Part model, mm, in its own coordinate system. Round coordinates to 2 decimals unless told otherwise and drop trailing zeros. Loops run counter-clockwise (first coordinate to the right, second up) from the corner with the lowest first, then second, coordinate; pieces in that order, holes last.
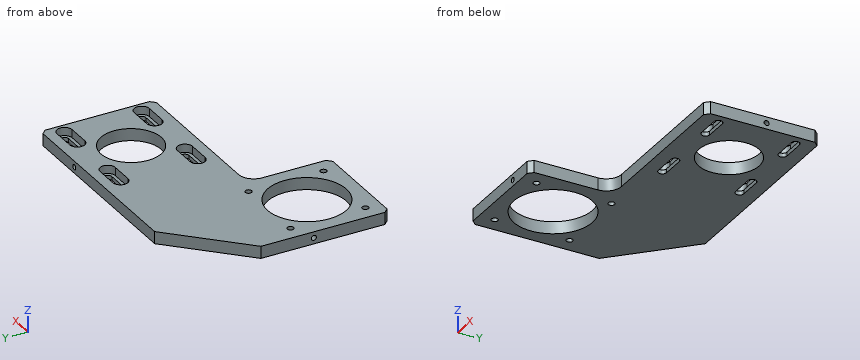
from build123d import *

# Parameters (mm, degrees)
SKETCH_2_W                     = 180
SKETCH_2_H                     = 130
EXTRUDE_1_DEPTH                = 4
SKETCH_3_W                     = 110
SKETCH_3_H                     = 55
CUT_EXTRUDE_1_DEPTH            = 8
SKETCH_4_R                     = 26
CUT_EXTRUDE_2_DEPTH            = 8
HOLE_WIZARD_M5_1_D             = 4.2
HOLE_WIZARD_M5_1_DEPTH         = 12.4
HOLE_WIZARD_M5_1_TIP           = 1.2618073
SKETCH_7_R                     = 20
CUT_EXTRUDE_3_DEPTH            = 8
HOLE_WIZARD_M4_1_D             = 3.3
HOLE_WIZARD_M4_1_DEPTH         = 12
HOLE_WIZARD_M4_1_TIP           = 0.991420021
HOLE_WIZARD_M4_2_D             = 3.3
HOLE_WIZARD_M4_2_DEPTH         = 12
HOLE_WIZARD_M4_2_TIP           = 0.991420021
CHAMFER_1_SIZE                 = 45
CHAMFER_2_SIZE                 = 3
FILLET_1_R                     = 10
HOLE_WIZARD_M5_1_2_D           = 5.5
HOLE_WIZARD_M5_1_2_DEPTH       = 10.1
HOLE_WIZARD_M5_1_2_CBORE_D     = 10
HOLE_WIZARD_M5_1_2_CBORE_DEPTH = 5.4
HOLE_WIZARD_M5_1_2_TIP         = 1.652366702
CUT_EXTRUDE_6_DEPTH            = 112.30588484
CUT_EXTRUDE_7_DEPTH            = 5.4
PATTERN_LINEAR_1_COUNT         = 2
PATTERN_LINEAR_1_PITCH         = 51
PATTERN_LINEAR_1_COUNT_DIR2    = 2
PATTERN_LINEAR_1_PITCH_DIR2    = 51
HOLE_WIZARD_M4_3_D             = 3.3
HOLE_WIZARD_M4_3_DEPTH         = 10.1
HOLE_WIZARD_M4_3_TIP           = 0.991420021
HOLE_WIZARD_M4_4_D             = 3.3
HOLE_WIZARD_M4_4_DEPTH         = 10.1
HOLE_WIZARD_M4_4_TIP           = 0.991420021


with BuildPart() as part:
    # 草图2 → 凸台-拉伸1 (new, symmetric)
    with BuildSketch(Plane.XY):
        Rectangle(SKETCH_2_W, SKETCH_2_H)
    extrude(amount=EXTRUDE_1_DEPTH, both=True)

    # 草图3 → 切除-拉伸1 (cut)
    with BuildSketch(Plane.XY.offset(4)):
        with Locations((35, -37.5)):
            Rectangle(SKETCH_3_W, SKETCH_3_H)
    extrude(amount=-CUT_EXTRUDE_1_DEPTH, mode=Mode.SUBTRACT)

    # 草图4 → 切除-拉伸2 (cut)
    with BuildSketch(Plane.XY.offset(4)):
        with Locations((-55, -30)):
            Circle(SKETCH_4_R)
    extrude(amount=-CUT_EXTRUDE_2_DEPTH, mode=Mode.SUBTRACT)

    # Hole Wizard M5 _1
    with Locations(Plane.XY.offset(4)):
        with Locations((-30.251262658, -54.748737342), (-79.748737342, -5.251262658), (-79.748737342, -54.748737342), (-30.251262658, -5.251262658)):
            Hole(HOLE_WIZARD_M5_1_D / 2, depth=HOLE_WIZARD_M5_1_DEPTH)
            with Locations((0, 0, -(HOLE_WIZARD_M5_1_DEPTH + HOLE_WIZARD_M5_1_TIP / 2))):  # 118° drill point
                Cone(0, HOLE_WIZARD_M5_1_D / 2, HOLE_WIZARD_M5_1_TIP, mode=Mode.SUBTRACT)

    # 草图7 → 切除-拉伸3 (cut)
    with BuildSketch(Plane.XY.offset(4)):
        with Locations((50, 27.5)):
            Circle(SKETCH_7_R)
    extrude(amount=-CUT_EXTRUDE_3_DEPTH, mode=Mode.SUBTRACT)

    # M4 螺纹孔1
    with Locations(Plane(origin=(0, 65, 0), x_dir=(1, 0, 0), z_dir=(0, 1, 0))):
        with Locations((50, 0)):
            Hole(HOLE_WIZARD_M4_1_D / 2, depth=HOLE_WIZARD_M4_1_DEPTH)
            with Locations((0, 0, -(HOLE_WIZARD_M4_1_DEPTH + HOLE_WIZARD_M4_1_TIP / 2))):  # 118° drill point
                Cone(0, HOLE_WIZARD_M4_1_D / 2, HOLE_WIZARD_M4_1_TIP, mode=Mode.SUBTRACT)

    # M4 螺纹孔2
    with Locations(Plane(origin=(0, -65, 0), x_dir=(-1, 0, 0), z_dir=(0, -1, 0))):
        with Locations((40, 0)):
            Hole(HOLE_WIZARD_M4_2_D / 2, depth=HOLE_WIZARD_M4_2_DEPTH)
            with Locations((0, 0, -(HOLE_WIZARD_M4_2_DEPTH + HOLE_WIZARD_M4_2_TIP / 2))):  # 118° drill point
                Cone(0, HOLE_WIZARD_M4_2_D / 2, HOLE_WIZARD_M4_2_TIP, mode=Mode.SUBTRACT)

    # 倒角1
    chamfer_1_edges = [part.edges().sort_by_distance(p)[0] for p in [
        (-90, 65, 0),
    ]]
    chamfer(chamfer_1_edges, length=CHAMFER_1_SIZE)

    # 倒角2
    chamfer_2_edges = [part.edges().sort_by_distance(p)[0] for p in [
        (90, -10, 0),
        (-20, -65, 0),
        (-90, -65, 0),
        (90, 65, 0),
    ]]
    chamfer(chamfer_2_edges, length=CHAMFER_2_SIZE)

    # 圆角1
    fillet_1_edges = [part.edges().sort_by_distance(p)[0] for p in [
        (-20, -10, 0),
    ]]
    fillet(fillet_1_edges, radius=FILLET_1_R)

    # Hole Wizard M5 _1 2
    with Locations(Plane.XY.offset(4)):
        with Locations((24.5, 53), (75.5, 53), (24.5, 2), (75.5, 2)):
            CounterBoreHole(HOLE_WIZARD_M5_1_2_D / 2, HOLE_WIZARD_M5_1_2_CBORE_D / 2, HOLE_WIZARD_M5_1_2_CBORE_DEPTH, depth=HOLE_WIZARD_M5_1_2_DEPTH)
            with Locations((0, 0, -(HOLE_WIZARD_M5_1_2_DEPTH + HOLE_WIZARD_M5_1_2_TIP / 2))):  # 118° drill point
                Cone(0, HOLE_WIZARD_M5_1_2_D / 2, HOLE_WIZARD_M5_1_2_TIP, mode=Mode.SUBTRACT)

    # 草图18 → 切除-拉伸6 (cut, through all)
    with BuildSketch(Plane.XY.offset(4)):
        with BuildLine():
            Line((17, 55.75), (32, 55.75))
            ThreePointArc((32, 55.75), (34.75, 53), (32, 50.25))
            Line((32, 50.25), (17, 50.25))
            ThreePointArc((17, 50.25), (14.25, 53), (17, 55.75))
        make_face()
    cut_extrude_6 = extrude(amount=-CUT_EXTRUDE_6_DEPTH, mode=Mode.SUBTRACT)

    # 草图19 → 切除-拉伸7 (cut)
    with BuildSketch(Plane.XY.offset(4)):
        with BuildLine():
            Line((17, 58), (32, 58))
            ThreePointArc((32, 58), (37, 53), (32, 48))
            Line((32, 48), (17, 48))
            ThreePointArc((17, 48), (12, 53), (17, 58))
        make_face()
    cut_extrude_7 = extrude(amount=-CUT_EXTRUDE_7_DEPTH, mode=Mode.SUBTRACT)

    # 阵列(线性)1: 切除-拉伸6, Cut-Extrude 7 2 × 2
    with Locations(*[(i * PATTERN_LINEAR_1_PITCH, -j * PATTERN_LINEAR_1_PITCH_DIR2, 0) for i in range(PATTERN_LINEAR_1_COUNT) for j in range(PATTERN_LINEAR_1_COUNT_DIR2) if (i, j) != (0, 0)]):
        add(cut_extrude_6, mode=Mode.SUBTRACT)
        add(cut_extrude_7, mode=Mode.SUBTRACT)

    # M4 螺纹孔3
    with Locations(Plane.ZY.offset(90)):
        with Locations((0, -15)):
            Hole(HOLE_WIZARD_M4_3_D / 2, depth=HOLE_WIZARD_M4_3_DEPTH)
            with Locations((0, 0, -(HOLE_WIZARD_M4_3_DEPTH + HOLE_WIZARD_M4_3_TIP / 2))):  # 118° drill point
                Cone(0, HOLE_WIZARD_M4_3_D / 2, HOLE_WIZARD_M4_3_TIP, mode=Mode.SUBTRACT)

    # M4 螺纹孔4
    with Locations(Plane(origin=(90, 0, 0), x_dir=(0, 0, -1), z_dir=(1, 0, 0))):
        with Locations((0, 30)):
            Hole(HOLE_WIZARD_M4_4_D / 2, depth=HOLE_WIZARD_M4_4_DEPTH)
            with Locations((0, 0, -(HOLE_WIZARD_M4_4_DEPTH + HOLE_WIZARD_M4_4_TIP / 2))):  # 118° drill point
                Cone(0, HOLE_WIZARD_M4_4_D / 2, HOLE_WIZARD_M4_4_TIP, mode=Mode.SUBTRACT)


solid = part.part
1) Slice it at C-C, the plane y = 2.5. Give the cut face in (x, z), then the cut area to 3 significant figures.
Values:
outline: (-90, -4) - (14.3, -4) - (14.3, -1.4) - (12.03, -1.4) - (12.03, 4) - (-90, 4) - close; (34.7, -4) - (65.3, -4) - (65.3, -1.4) - (63.03, -1.4) - (63.03, 4) - (36.97, 4) - (36.97, -1.4) - (34.7, -1.4) - close; (85.7, -4) - (90, -4) - (90, 4) - (87.97, 4) - (87.97, -1.4) - (85.7, -1.4) - close
area: 1,060 mm2
2) Wall check: line 1 along Y through (x, z) = (78.5, -1); line 2 along Z through (x, y) = (-85.25, -15); line 3 along Y through (x, z) = (-31, -1). Give the ranges that are in metal, low to high.
Values:
line 1: y = -10 to -3, 7 to 48, 58 to 65
line 2: z = -4 to -1.65, 1.65 to 4
line 3: y = -65 to -56.71, -52.79 to -40, -20 to -7.21, -3.29 to 65
3) Drop flat-ended pins along their axis: pin 1 Ø4 at (y, z) = (-33.5, 1) entering from +X; pin 2 Ø1.6 at (x, z) = (72, 0.5) entering from -Y; pin 3 Ø4 at (y, z) = (30, 0) entering from -X. Give the stop position or say it passes through.
Values:
pin 1: stops at x = -20
pin 2: stops at y = -10
pin 3: stops at x = -82
4) Slice it at A-A, the plane y = -30. Give the cut face in (x, z).
Values:
outline: (-90, -4) - (-81, -4) - (-81, 4) - (-90, 4) - close; (-29, -4) - (-20, -4) - (-20, 4) - (-29, 4) - close
5) Slice it at B-B, the plane x = 44. Give the cut face in (y, z), then the cut area to 3 significant figures.
Values:
outline: (-10, -4) - (8.42, -4) - (8.42, 4) - (-10, 4) - close; (46.58, -4) - (65, -4) - (65, 4) - (46.58, 4) - close
area: 295 mm2
